The listing builds one solid part. Answer for the finished solid, in the listing's coordinates (mm). Face numbers are marked on the shaded views. A direction names the side the tool comes from. Round coordinates to 2 decimals unless told otherwise and drop trailing zeros. Loops run counter-clockwise (first coordinate to the right, second up) from the corner with the lowest first, then second, coordinate; pieces in that order, holes last. Notation, with made-up numbers: (47.5, 11) - (75.5, 11) arc R25 ccw to (75.5, 32) - close; hole circle Ø3 at (-11, -23). An arc over 180 degrees is marked (long way). Write item = value, one per line. Start each with the question number.
1) Section B-B, the plane z = -7 is taken. Determine the outline of the cut face in (x, y).
2) Section D-D, the plane x = -113.5 is taken. Determine the outline of the cut face in (y, z), and give its area (3 significant figures).
3) Given pin 1 Ø5 at (y, z) = (-35.5, 10) entering from -X; pin 2 Ø4 at (y, z) = (10, 3) entering from -X, each flat-ended and moving along its own axis, determine where each tip first touches the part or whether it passes through.
4) Section A-A, the plane x = 0 is taken. Determine the outline of the cut face in (y, z), and give its area (4 significant figures).
5) Straight lines are drawn through the part: line 1 along Y through (x, z) = (0, 5.5); line 2 along X through (y, z) = (-5, -1.5); line 3 along Y through (x, z) = (-191.5, 10.5). For each, find the intervals that lie inside material, in ascending order.
6) Section C-C, the plane y = 0 is taken. Determine the outline of the cut face in (x, z).
7) A tool of negligible diameter and unlimited length cuts with its end or side. For the marked faces 5, 6 and 7, from which of +Z, -Z, +X, -X, +Y, -Y can it reach the whole face along a straight path? Write none if from no direction.
8) For a pull along Y with two mould halves and no side action, classify the marked faces 1, 2, 3 and 4 as released by +Y, released by -Y, zero draft, split by the parting line, or undercut.
from build123d import *

# Parameters (mm, degrees)
SKETCH1_R           = 40
BOSS_EXTRUDE1_DEPTH = 25
CHAMFER1_SIZE       = 15


with BuildPart() as part:
    # Sketch1 → Boss-Extrude1 (new, symmetric)
    with BuildSketch(Plane.XY):
        with BuildLine():
            Line((-280, 105), (280, 105))
            Line((280, 105), (280, 85))
            Line((280, 85), (173.275566379, 47.11998854))
            ThreePointArc((173.275566379, 47.11998854), (140, 0), (173.275566379, -47.11998854))
            Line((173.275566379, -47.11998854), (280, -85))
            Line((280, -85), (280, -105))
            Line((280, -105), (-280, -105))
            Line((-280, -105), (-280, -85))
            Line((-280, -85), (-173.275566379, -47.11998854))
            ThreePointArc((-173.275566379, -47.11998854), (-140, 0), (-173.275566379, 47.11998854))
            Line((-173.275566379, 47.11998854), (-280, 85))
            Line((-280, 85), (-280, 105))
        make_face()
        Circle(SKETCH1_R, mode=Mode.SUBTRACT)
    extrude(amount=BOSS_EXTRUDE1_DEPTH, both=True)

    # Chamfer1
    chamfer1_edges = [part.edges().sort_by_distance(p)[0] for p in [
        (0, 105, 25),
        (0, -105, 25),
    ]]
    chamfer(chamfer1_edges, length=CHAMFER1_SIZE)


solid = part.part
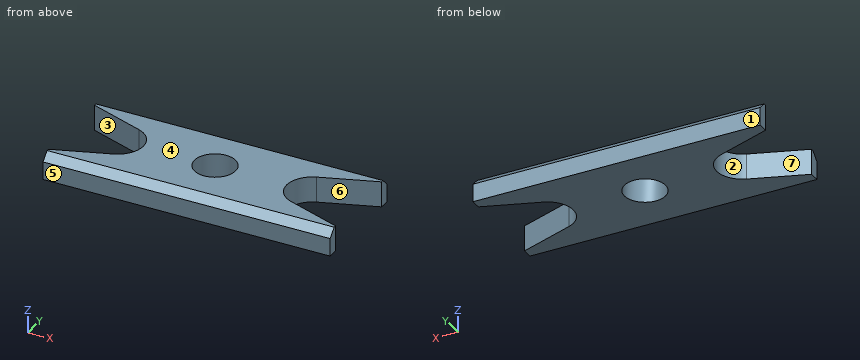
Geometry check:
q1.outline = (-280, -105) - (280, -105) - (280, -85) - (173.28, -47.12) arc R50 cw to (173.28, 47.12) - (280, 85) - (280, 105) - (-280, 105) - (-280, 85) - (-173.28, 47.12) arc R50 cw to (-173.28, -47.12) - (-280, -85) - close; hole circle Ø80 at (0, 0)
q2.outline = (-105, -25) - (105, -25) - (105, 10) - (90, 25) - (-90, 25) - (-105, 10) - close
q2.area = 10,300 mm2
q3.pin_1 = -157.5
q3.pin_2 = -141.46
q4.outline = (-105, -25) - (-40, -25) - (-40, 25) - (-90, 25) - (-105, 10) - close; (40, -25) - (105, -25) - (105, 10) - (90, 25) - (40, 25) - close
q4.area = 6,275 mm2
q5.line_1 = -105 to -40, 40 to 105
q5.line_2 = -140.25 to -39.69, 39.69 to 140.25
q5.line_3 = -104.5 to -53.59, 53.59 to 104.5
q6.outline = (-140, -25) - (-40, -25) - (-40, 25) - (-140, 25) - close; (40, -25) - (140, -25) - (140, 25) - (40, 25) - close
q7.face_5 = +Z, -Z, +X, -X, -Y
q7.face_6 = +Z, -Z, +X
q7.face_7 = +Z, -Z, -X
q8.face_1 = released by +Y
q8.face_2 = undercut
q8.face_3 = undercut
q8.face_4 = zero draft
